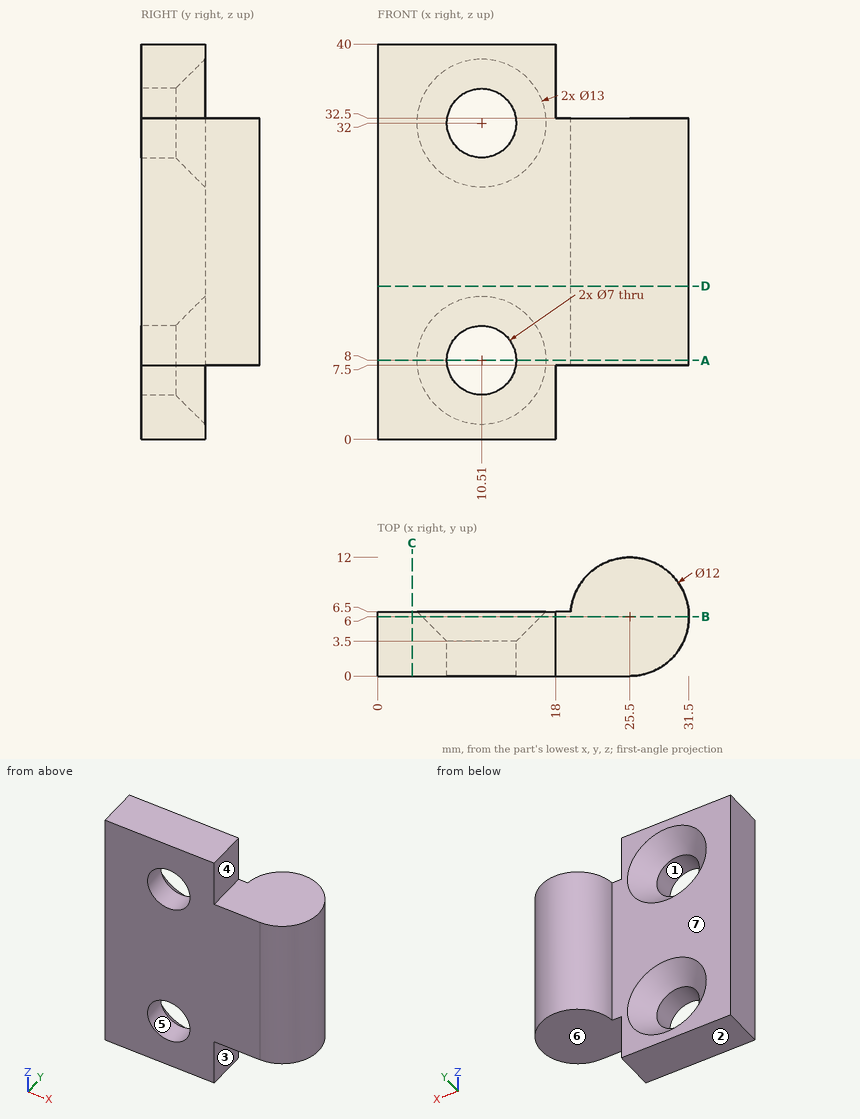
Part print with two shaded views. Sizes in mm from the minimum x, y, z corner. A direction names the side the tool comes from. Give positions to 0.01 mm unless a question says otherwise; leave off trailing zeros. Order: outer loops, then holes, each group sorted by start corner. A loop starts at its lowest first (then second) coordinate and runs counter-clockwise, first axis right, second up.
(1) Saw through at D-D, the plane z = 15.5. Give the cut face in (x, y).
(2) Saw through at A-A, the plane z = 8. Give the cut face in (x, y).
(3) Flat gauge pins, fed straight in: pin 1 (5 mm diameter, centred on x = 10, z = 28, fed in from +Y); pin 2 (3.5 mm diameter, centred on x = 23, y = 8, fed in from +Z); pin 3 (3 mm diameter, centred on y = 8, z = 18.5, fed in from +X). Where does each tip first touch, or does it go through?
(4) Saw through at B-B, the plane y = 6. Give the cut face in (x, z), then the cut area to 3 significant figures.
(5) Saw through at C-C, the plane x = 3.5. Give the cut face in (y, z), then the cut area to 3 significant figures.
(6) Mould opens along X. For the marked faces 1, 2 and 3 say: released by +X, released by -X, zero draft, split by the parting line, or undercut.
(7) Tool access for the marked faces 4, 5, 6 and 7: list every direction of +Z, -Z, +X, -X, +Y, -Y with a clear straight run to the whole face (end or side of a thin tool).
(8) Drill centre lines: L1, parallel to Y at x = 3.5, z = 11; L2, parallel to X at y = 2.7, z = 8; L3, parallel to X at y = 1.65, z = 32 (1 decimal). Where is each one in solid material? Low to high.
Results found:
1. outline: (0, 0) - (25.5, 0) arc R6 ccw (long way) to (19.52, 6.5) - (0, 6.5) - close
2. outline: (0, 0) - (7.01, 0) - (7.01, 3.5) - (4.01, 6.5) - (0, 6.5) - close; (14.01, 0) - (25.5, 0) arc R6 ccw (long way) to (19.52, 6.5) - (17.01, 6.5) - (14.01, 3.5) - close
3. pin 1: stops at y = 6.5
3. pin 2: stops at z = 32.5
3. pin 3: stops at x = 31.48
4. outline: (0, 0) - (18, 0) - (18, 7.5) - (31.5, 7.5) - (31.5, 32.5) - (18, 32.5) - (18, 40) - (0, 40) - close; hole circle Ø12 at (10.51, 8); hole circle Ø12 at (10.51, 32)
4. area: 831 mm2
5. outline: (0, 0) - (6.5, 0) - (6.5, 40) - (0, 40) - close
5. area: 260 mm2
6. face 1: undercut
6. face 2: zero draft
6. face 3: released by +X
7. face 4: +Z, +X, +Y, -Y
7. face 5: +Y, -Y
7. face 6: -Z, +X, +Y, -Y
7. face 7: +Z, -Z, -X, +Y
8. L1: y = 0 to 6.5
8. L2: x = 0 to 7.01, 14.01 to 30.51
8. L3: x = 0 to 7, 14 to 29.6
